Source: three-view drawing plus pictorial views. Frame: mm from the lowest corner of the part. Coordinates: 2 decimals unless noted, no trailing zeros. Write each loop counter-clockwise with the first axis right and the second up, starting at its lowest first coordinate (ties: lowest second). Pieces come first, ordered by that corner, then holes. Notation, with made-up numbers: (3, 21.25) -> (18, 21.25) arc R8 ccw to (18, 31.25) -> close; hole circle Ø3 at (32, 6). An arc over 180 degrees is marked (long way). One line per item, written item: value.
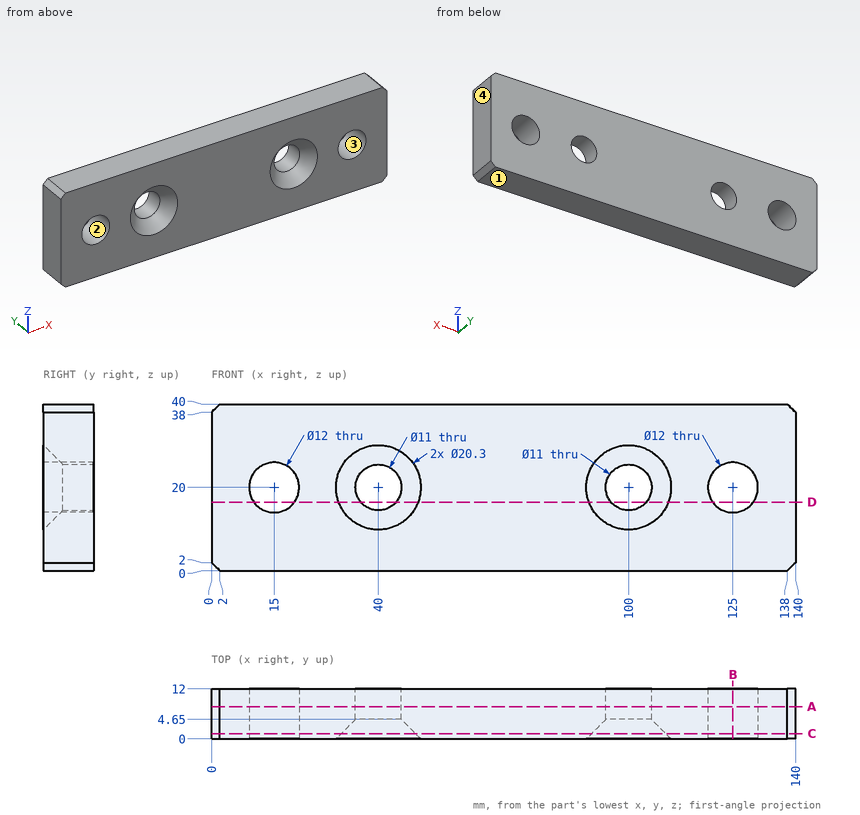
(1) Section D-D (z = 16.5). State how many separate pieces and enclosed holes the cut face has, then the cut area to 3 significant figures.
Responses:
separate pieces: 5
enclosed holes: 0
area: 1,190 mm2
(2) Pull-direction query (Z, two-part tool) for the marked faces 1, 2, 3 and 4; classes: released by +Z, released by -Z, zero draft, split by the parting line, or undercut.
Responses:
face 1: released by -Z
face 2: undercut
face 3: undercut
face 4: zero draft
(3) Section A-A (y = 7.75). Return the cut outline in (x, z).
Responses:
outline: (0, 2) -> (2, 0) -> (138, 0) -> (140, 2) -> (140, 38) -> (138, 40) -> (2, 40) -> (0, 38) -> close; hole circle Ø12 at (15, 20); hole circle Ø11 at (40, 20); hole circle Ø11 at (100, 20); hole circle Ø12 at (125, 20)
(4) First-contact query: pin 1 (3 mm diameter, centred on x = 16, z = 22.5, fed in from +Y); pin 2 (14.5 mm diameter, centred on x = 100, z = 20, fed in from -Y). Flat tips, straight axial feed; report the tip coordinate or a pass-through.
Responses:
pin 1: passes through
pin 2: stops at y = 2.9
(5) Section C-C (y = 1.25). Return the cut outline in (x, z), then the cut area to 3 significant figures.
Responses:
outline: (0, 2) -> (2, 0) -> (138, 0) -> (140, 2) -> (140, 38) -> (138, 40) -> (2, 40) -> (0, 38) -> close; hole circle Ø12 at (15, 20); hole circle Ø17.8 at (40, 20); hole circle Ø17.8 at (100, 20); hole circle Ø12 at (125, 20)
area: 4,870 mm2
(6) Section B-B (x = 125). Return the cut outline in (y, z), then the cut area to 3 significant figures.
Responses:
outline: (0, 0) -> (12, 0) -> (12, 14) -> (0, 14) -> close; (0, 26) -> (12, 26) -> (12, 40) -> (0, 40) -> close
area: 336 mm2
(7) Line query: line 1 (X direction, y = 7.25, z = 20); line 2 (Z direction, x = 40, y = 10.5); line 3 (Z direction, x = 125, y = 8.5). Output: solid intervals per line, ascending. Write a range as [from, to].
Responses:
line 1: x = [0, 9], [21, 34.5], [45.5, 94.5], [105.5, 119], [131, 140]
line 2: z = [0, 14.5], [25.5, 40]
line 3: z = [0, 14], [26, 40]
